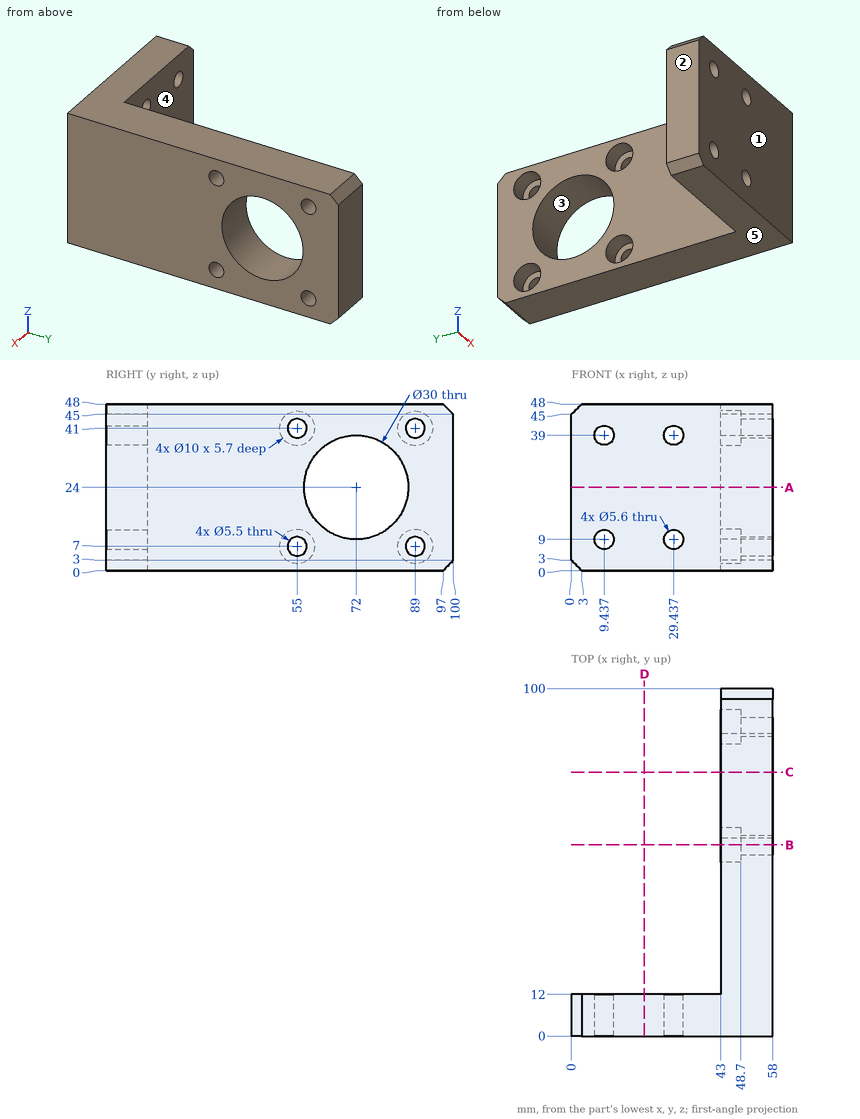
Input: dimensioned drawing with shaded views. Units: mm. Origin: part minimum x, y, z. A direction names the side the tool comes from. Give positions to 0.01 mm unless a question says otherwise; leave off trailing zeros. Write each loop counter-clockwise with the first axis right and the second up, starting at its lowest first coordinate (ties: lowest second). Pieces come first, ordered by that corner, then holes.
1. First-contact query: pin 1 (8 mm diameter, centred on y = 54, z = 40.5, fed in from -X); pin 2 (6 mm diameter, centred on y = 55, z = 41, fed in from -X); pin 3 (21.5 mm diameter, centred on x = 14.5, z = 17, fed in from +Y). Flat tips, straight axial feed; report the tip coordinate or a pass-through.
2. Access query for the marked faces 4 and 5. Directions: +Z, -Z, +X, -X, +Y, -Y. A direction counts if a zero-diameter tool reaches every point of the face in a straight line with its end or side. Return the directions, or none.
3. Section query A-A (z = 24). Return the cut outline in (x, y), then the cut area to 3 significant figures.
4. Material intervals for line 1 along Z through (x, y) = (53, 89); line 2 along Y through (x, z) = (52, 7); line 3 along X through (y, z) = (43, 33.5), sorted ascending.
5. Section query B-B (y = 55). Return the cut outline in (x, z).
6. Section query D-D (x = 21). Return the cut outline in (y, z), then the cut area to 3 significant figures.
7. Pull-direction query (Y, two-part tool) for the marked faces 1, 2 and 3; classes: +Y half, -Y half, draft (parallel to the pull), parting line (faces both ways), or undercut.
8. Section query C-C (y = 76). Return the cut outline in (x, z), then the cut area to 3 significant figures.
Output values:
1. pin 1: stops at x = 43
1. pin 2: stops at x = 48.7
1. pin 3: stops at y = 12
2. face 4: +Z, -Z, -X, +Y
2. face 5: -Z, +X, -X, +Y, -Y
3. outline: (0, 0) - (58, 0) - (58, 57) - (43, 57) - (43, 12) - (0, 12) - close; (43, 87) - (58, 87) - (58, 100) - (43, 100) - close
3. area: 1,570 mm2
4. line 1: z = 0 to 4.25, 9.75 to 38.25, 43.75 to 48
4. line 2: y = 0 to 52.25, 57.75 to 86.25, 91.75 to 100
4. line 3: x = 43 to 58
5. outline: (43, 0) - (58, 0) - (58, 4.25) - (48.7, 4.25) - (48.7, 2) - (43, 2) - close; (43, 12) - (48.7, 12) - (48.7, 9.75) - (58, 9.75) - (58, 38.25) - (48.7, 38.25) - (48.7, 36) - (43, 36) - close; (43, 46) - (48.7, 46) - (48.7, 43.75) - (58, 43.75) - (58, 48) - (43, 48) - close
6. outline: (0, 0) - (12, 0) - (12, 48) - (0, 48) - close
6. area: 576 mm2
7. face 1: -Y half
7. face 2: draft
7. face 3: undercut
8. outline: (43, 0) - (58, 0) - (58, 9.54) - (43, 9.54) - close; (43, 38.46) - (58, 38.46) - (58, 48) - (43, 48) - close
8. area: 286 mm2
